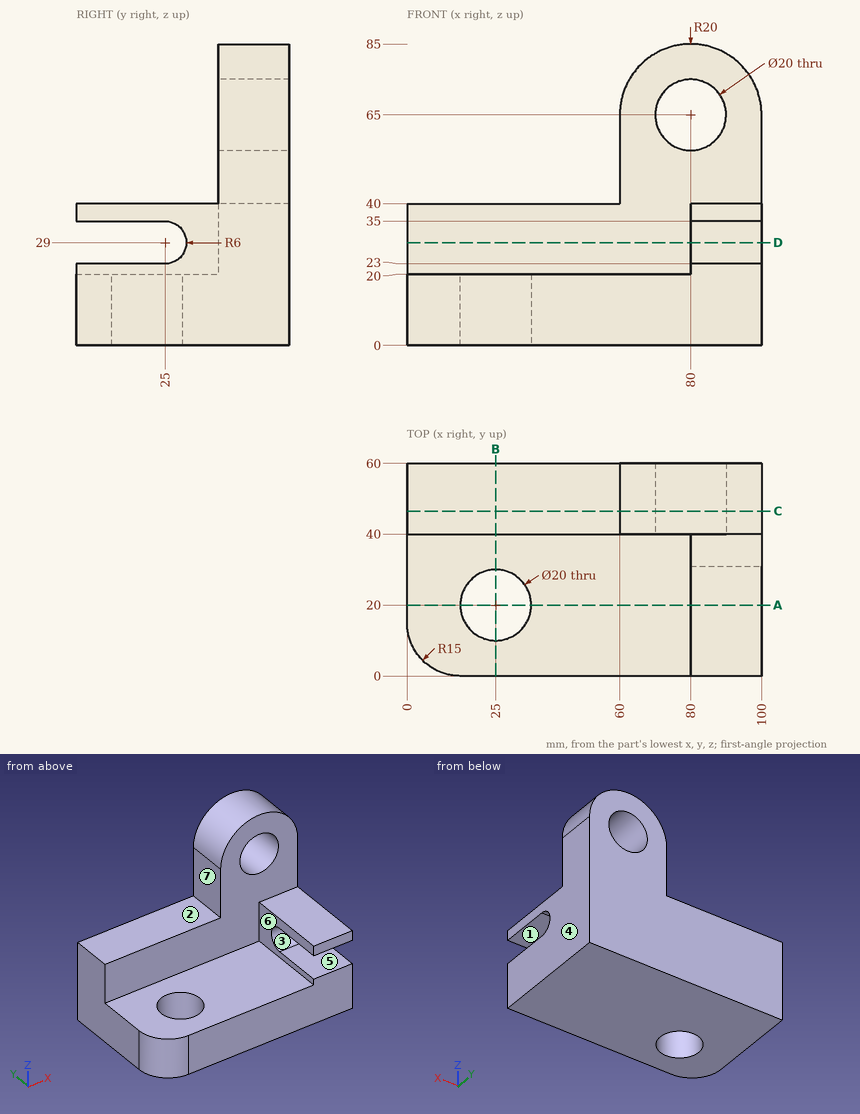
Design review of the part shown in the three views and the two pictorial views. Dimensions are in mm from the part's minimum x, y and z. A direction names the side the tool comes from. Coordinates: 2 decimals unless noted, no trailing zeros. Order: outer loops, then holes, each group sorted by start corner. A loop starts at its lowest first (then second) coordinate and runs counter-clockwise, first axis right, second up.
Item 1: Take a section at C-C, the plane y = 46.5. Write out the cut boundary in (x, z), then the cut area to 3 significant figures.
Item 2: Take a section at D-D, the plane z = 29. Write out the cut boundary in (x, y).
Item 3: For line 1 (Y direction, x = 25, z = 4.75); line 2 (Z direction, x = 83.5, y = 19.5); line 3 (X direction, y = 56, z = 65), list the stretches that pass through material, from the lowest coordinate up.
Item 4: Take a section at B-B, the plane x = 25. Write out the cut boundary in (y, z).
Item 5: For pin 1 Ø6 at (x, y) = (92, 8.5) entering from +Z; pin 2 Ø22 at (y, z) = (53, 58.5) entering from -X; pin 3 Ø12 at (x, y) = (31.5, 12) entering from +Z, all flat-tipped, find the tip position at first contact; note any pin that passes through.
Item 6: Take a section at A-A, the plane y = 20. Write out the cut boundary in (x, z).
Item 7: The part is to be moulded in two halves that separate along Z. For the marked faces 1, 2, 3 and 4, say which applies: pulls with the +Z half, pulls with the -Z half, needs draft (parallel to the pull), parting line crosses it, or undercut.
Item 8: For the marked faces 5, 6 and 7, list the 3-axis set-ups (+Z, -Z, +X, -X, +Y, -Y) from which the entire face can be reached by the end or side of a thin tool; tool diameter is ignored.
The answers:
1. outline: (0, 0) - (100, 0) - (100, 65) arc R20 ccw to (60, 65) - (60, 40) - (0, 40) - close; hole circle Ø20 at (80, 65)
1. area: 5,310 mm2
2. outline: (0, 40) - (80, 40) - (80, 31) - (100, 31) - (100, 60) - (0, 60) - close
3. line 1: y = 0 to 10, 30 to 60
3. line 2: z = 0 to 23, 35 to 40
3. line 3: x = 60 to 70, 90 to 100
4. outline: (0, 0) - (10, 0) - (10, 20) - (0, 20) - close; (30, 0) - (60, 0) - (60, 40) - (40, 40) - (40, 20) - (30, 20) - close
5. pin 1: stops at z = 40
5. pin 2: stops at x = 60
5. pin 3: stops at z = 20
6. outline: (0, 0) - (15, 0) - (15, 20) - (0, 20) - close; (35, 0) - (100, 0) - (100, 23) - (80, 23) - (80, 20) - (35, 20) - close; (80, 35) - (100, 35) - (100, 40) - (80, 40) - close
7. face 1: undercut
7. face 2: pulls with the +Z half
7. face 3: undercut
7. face 4: needs draft
8. face 5: +X, -X, -Y
8. face 6: +Z, -X, -Y
8. face 7: +Z, -X, +Y, -Y
